Read the model definition and answer for the solid it produces. Units are mm, in the model's axes. A direction names the side the tool comes from. Coordinates: 2 decimals unless noted, no trailing zeros. Write each loop counter-clockwise with the first axis right and the second up, starting at its lowest first coordinate (ties: lowest second). Pieces come first, ordered by that corner, then holes. Notation, with made-up numbers: (83, 87.5) -> (138, 87.5) arc R20 ccw to (138, 99.5) -> close; hole circle Ø2 at (-28, 53.5). An arc over 180 degrees is marked (long way). Answer in a Markdown table with one row per item. Add a question column.
Item 1: Which of the six approach directions +Z, -Z, +X, -X, +Y, -Y give full straight-line access (tool end or side, diameter ignored) to faces 5 (the face through (1, 5, 3.923)), 6 (the face through (7.263, -0.018, 6.429)), 7 (the face through (4.64, 1.46, 21.51))?
Item 2: Straight lines are drawn through the part: line 1 (Z direction, x = 3, y = 4.5); line 2 (Y direction, x = 0, z = 6); line 3 (Y direction, x = 0, z = 22). For each, find the intervals that lie inside material, in ascending order. Write a range as from..to.
Item 3: Section B-B on z = 20.25 is taken. Write down the section's boundary in (x, y), then the cut area to 3 significant figures.
Item 4: For a pull along Z with two mould halves and no side action, classify faces 1 (the face through (2.58, 4.05, 2.96)), 2 (the face through (-4.21, -3.22, 4.12)), 3 (the face through (-3.64, -6.28, 17.85)), 4 (the face through (-0.703, -3.166, 21.19)) as +Z half, -Z half, draft (parallel to the pull), parting line (faces both ways), or undercut.
Item 5: Given pin 1 Ø4 at (x, y) = (-1.5, 0.5) entering from -Z, flat-ended and moving along its own axis, determine where the tip first touches the part or whether it passes through.
Item 6: Section A-A on z = 15.75 is taken. Write down the section's boundary in (x, y).
```python
from build123d import *

# Parameters (mm, degrees)
SKETCH_2_R          = 14
CUT_EXTRUDE_1_DEPTH = 25.5


with BuildPart() as part:
    # 草图1 → 旋转1 (revolve)
    with BuildSketch(Plane(origin=(0, 0, 0), x_dir=(0, 0, -1), z_dir=(1, 0, 0)), mode=Mode.PRIVATE) as revolve_1_sk:
        with BuildLine():
            Line((-25.5, 3.242666667), (-17, 3.242666667))
            Line((-17, 3.242666667), (-17, 4))
            Line((-17, 4), (0, 4))
            Line((0, 4), (0, 6.75))
            ThreePointArc((0, 6.75), (-0.073223305, 6.926776695), (-0.25, 7))
            Line((-0.25, 7), (-1.961538462, 7))
            Line((-1.961538462, 7), (-1.961538462, 4.8))
            Line((-1.961538462, 4.8), (-3.923076923, 4.8))
            Line((-3.923076923, 4.8), (-3.923076923, 5.3))
            Line((-3.923076923, 5.3), (-4.315384615, 5.3))
            ThreePointArc((-4.315384615, 5.3), (-4.608277834, 6.007106781), (-5.315384615, 6.3))
            Line((-5.315384615, 6.3), (-6.276923077, 6.3))
            Line((-6.276923077, 6.3), (-6.276923077, 7))
            Line((-6.276923077, 7), (-6.902137859, 8.082903769))
            Line((-6.902137859, 8.082903769), (-17.374785218, 8.082903769))
            Line((-17.374785218, 8.082903769), (-18, 7))
            Line((-18, 7), (-18, 4.864))
            Line((-18, 4.864), (-24.919, 4.864))
            Line((-24.919, 4.864), (-25.5, 4.283))
            Line((-25.5, 4.283), (-25.5, 3.242666667))
        make_face()
    revolve(revolve_1_sk.sketch.rotate(Axis((0, 0, 0), (0, 0, 1)), 270), axis=Axis((0, 0, 0), (0, 0, 1)))

    # 草图2 → 切除-拉伸1 (cut)
    with BuildSketch(Plane(origin=(0, 0, 6.276923077), x_dir=(-1, 0, 0), z_dir=(0, 0, -1))):
        Circle(SKETCH_2_R)
        Polygon((-4.041451884, -7), (4.041451884, -7), (8.082903769, 0), (4.041451884, 7), (-4.041451884, 7), (-8.082903769, 0), align=None, mode=Mode.SUBTRACT)
    extrude(amount=-CUT_EXTRUDE_1_DEPTH, mode=Mode.SUBTRACT)


solid = part.part
```
Results below:
| question | item | result |
|---|---|---|
| 1 | face 5 | none |
| 1 | face 6 | -Z, +X |
| 1 | face 7 | +Z |
| 2 | line 1 | z = 0..1.96, 4.32..18 |
| 2 | line 2 | y = -6.3..-4, 4..6.3 |
| 2 | line 3 | y = -4.86..-3.24, 3.24..4.86 |
| 3 | outline | circle Ø9.73 at (0, 0); hole circle Ø6.49 at (0, 0) |
| 3 | area | 41.3 mm2 |
| 4 | face 1 | undercut |
| 4 | face 2 | undercut |
| 4 | face 3 | +Z half |
| 4 | face 4 | draft |
| 5 | pin 1 | stops at z = 17 |
| 6 | outline | (-8.08, 0) -> (-4.04, -7) -> (4.04, -7) -> (8.08, 0) -> (4.04, 7) -> (-4.04, 7) -> close; hole circle Ø8 at (0, 0) |
